The listing builds one solid part. Answer for the finished solid, in the listing's coordinates (mm). Face numbers are marked on the shaded views. A direction names the side the tool comes from. Give positions to 0.01 mm unless a question says otherwise; leave off trailing zeros. Order: outer loops, then holes, each group sorted by start corner. A loop starts at its lowest first (then second) coordinate and runs counter-clockwise, first axis right, second up. Notation, with made-up numbers: (59, -22.75) - (77, -22.75) arc R34 ccw to (77, 15.25) - close; hole circle Ø5 at (47.5, 7). An arc over 180 degrees is marked (long way). Write each question's results on one line, items separated by ' | '. Start each with the question number.
1. Section C-C (x = -77.5) is taken. Give the vertices of the cut face in (y, z).
2. Flat-ended cylindrical pins translate along their axes: pin 1 (10 mm diameter, centred on x = -128, y = -49.5, fed in from +Z); pin 2 (10 mm diameter, centred on x = -138, y = 86, fed in from -Z). Find the tip coordinate at first contact, or state that the pin passes through.
3. Section A-A (y = 32) is taken. Give the vertices of the cut face in (x, z), and give its area (3 significant figures).
4. Determine the mould class of the marked faces 3, 4 and 5 for opening direction X: released by +X, released by -X, zero draft, split by the parting line, or undercut.
5. Which of the six approach directions +Z, -Z, +X, -X, +Y, -Y give full straight-line access (tool end or side, diameter ignored) to the marked faces 1 and 2?
6. Section B-B (z = 104) is taken. Give the vertices of the cut face in (x, y).
7. Find the intervals of material crossed by L1, parallel to Y at x = 142, z = 99; L2, parallel to X at y = -79.5, z = 35; L3, parallel to Z at x = 9, y = -43, in increasing order.
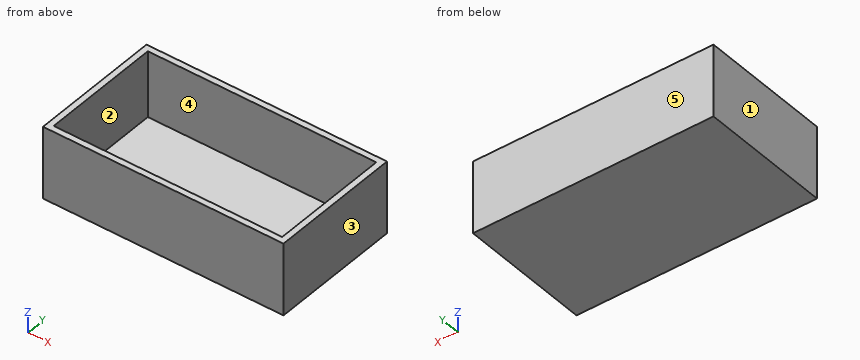
from build123d import *

# Parameters (mm, degrees)
SKETCH_1_W      = 400
SKETCH_1_H      = 220
SKETCH_1_W_2    = 380
SKETCH_1_H_2    = 200
EXTRUDE_1_DEPTH = 120
SKETCH_2_W      = 400
SKETCH_2_H      = 10
EXTRUDE_2_DEPTH = 210


with BuildPart() as part:
    # 草图1 → 拉伸-薄壁1 (new body)
    with BuildSketch(Plane.XY):
        Rectangle(SKETCH_1_W, SKETCH_1_H)
        Rectangle(SKETCH_1_W_2, SKETCH_1_H_2, mode=Mode.SUBTRACT)
    extrude(amount=EXTRUDE_1_DEPTH)

    # 草图2 → 凸台-拉伸2 (add)
    with BuildSketch(Plane(origin=(0, 100, 0), x_dir=(-1, 0, 0), z_dir=(0, -1, 0))):
        with Locations((0, -5)):
            Rectangle(SKETCH_2_W, SKETCH_2_H)
    extrude(amount=EXTRUDE_2_DEPTH)


solid = part.part
Reported:
1) outline: (-110, 0) - (110, 0) - (110, 120) - (100, 120) - (100, 10) - (-100, 10) - (-100, 120) - (-110, 120) - close
2) pin 1: z = 10 | pin 2: z = 0
3) outline: (-200, 0) - (200, 0) - (200, 120) - (190, 120) - (190, 10) - (-190, 10) - (-190, 120) - (-200, 120) - close | area: 6,200 mm²
4) face 3: released by +X | face 4: undercut | face 5: zero draft
5) face 1: +Z, -Z, -X, +Y, -Y | face 2: +Z
6) outline: (-200, -110) - (200, -110) - (200, 110) - (-200, 110) - close; hole (-190, -100) - (190, -100) - (190, 100) - (-190, 100) - close
7) L1: -110 to -100, 100 to 110 | L2: -200 to -190, 190 to 200 | L3: 0 to 10
